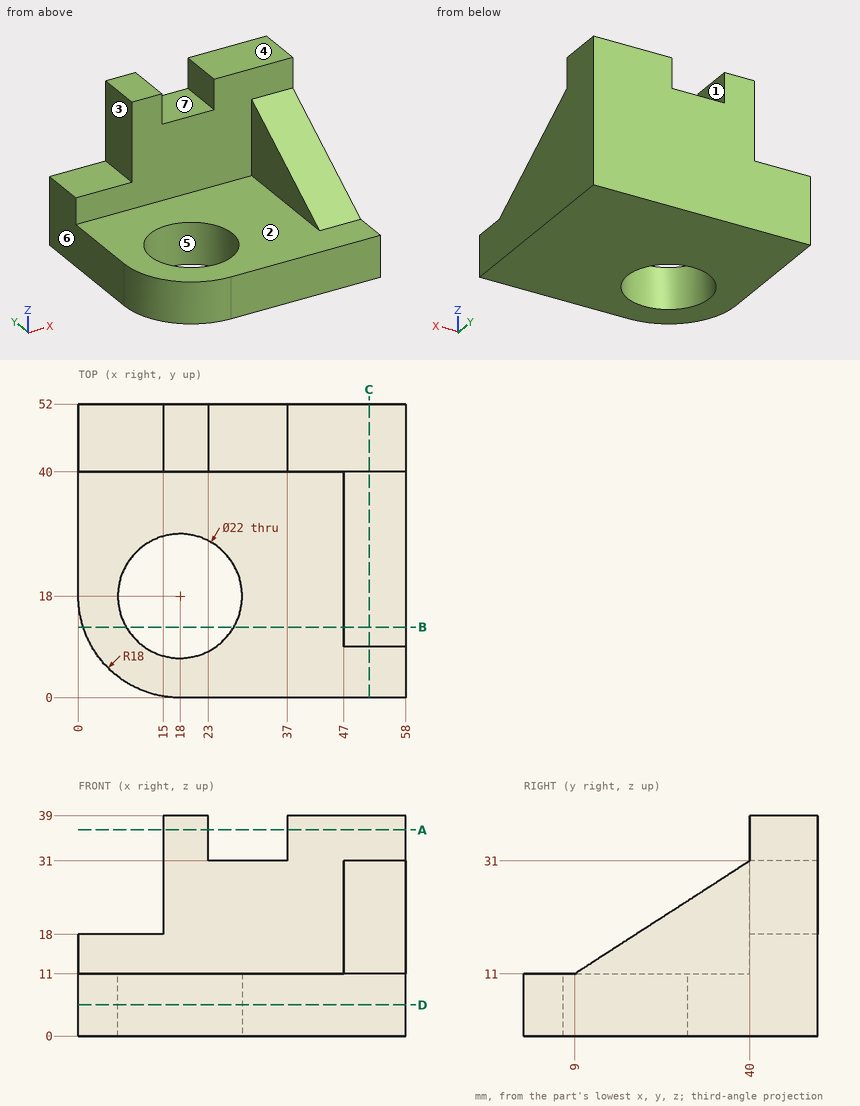
Geometry check sheet. Reference: drawing and pictorial views, mm from the part's lowest x, y, z. A direction names the side the tool comes from. Give positions to 0.01 mm unless a question says otherwise; leave off trailing zeros. Order: outer loops, then holes, each group sorted by start corner. A loop starts at its lowest first (then second) coordinate and runs counter-clockwise, first axis right, second up.
1. Section check D-D, the plane z = 5.5. Enter the section's corners in (x, y).
2. Release check for a two-part mould opening along X. For the marked faces 4, 5, 6 and 7 record: pulls with the +X half, pulls with the -X half, needs draft (parallel to the pull), parting line crosses it, or undercut.
3. Section check A-A, the plane z = 36.5. Enter the section's corners in (x, y), and give its area (3 significant figures).
4. Access from +Z, -Z, +X, -X, +Y, -Y to the whole of each face (thin tool, end or side, straight path). Record for the marked faces 1, 2 and 3.
5. Gauge pin test, flat ends, axial feed: pin 1 Ø3.5 at (x, y) = (6.5, 44) entering from +Z; pin 2 Ø16 at (y, z) = (20, 19.5) entering from -X; pin 3 Ø14 at (x, z) = (22.5, 29) entering from -Y. Record the tip position at first contact, or that the pin passes through.
6. Section check B-B, the plane y = 12.5. Enter the section's corners in (x, z), and give its area (3 significant figures).
7. Thickness scan on L1, parallel to Y at x = 18, z = 4.75; L2, parallel to Y at x = 39, z = 28; L3, parallel to X at y = 43, z = 24.5. Record the ranges inside material, lowest first.
8. Section check C-C, the plane x = 51.5. Enter the section's corners in (y, z), and give its area (3 significant figures).
Values follow:
1. outline: (0, 18) arc R18 ccw to (18, 0) - (58, 0) - (58, 52) - (0, 52) - close; hole circle Ø22 at (18, 18)
2. face 4: needs draft
2. face 5: undercut
2. face 6: pulls with the -X half
2. face 7: undercut
3. outline: (15, 40) - (23, 40) - (23, 52) - (15, 52) - close; (37, 40) - (58, 40) - (58, 52) - (37, 52) - close
3. area: 348 mm2
4. face 1: +Z, +Y, -Y
4. face 2: +Z, -X, -Y
4. face 3: +Z, -X, +Y, -Y
5. pin 1: stops at z = 18
5. pin 2: stops at x = 47
5. pin 3: stops at y = 40
6. outline: (0.86, 0) - (8.47, 0) - (8.47, 11) - (0.86, 11) - close; (27.53, 0) - (58, 0) - (58, 13.26) - (47, 13.26) - (47, 11) - (27.53, 11) - close
6. area: 444 mm2
7. L1: y = 0 to 7, 29 to 52
7. L2: y = 40 to 52
7. L3: x = 15 to 58
8. outline: (0, 0) - (52, 0) - (52, 39) - (40, 39) - (40, 31) - (9, 11) - (0, 11) - close
8. area: 1,220 mm2
